from build123d import *

# Parameters (mm, degrees)
LUG_PLATE_PROFILE_SKETCH_R   = 7.5
LUG_PLATE_PROFILE_14MM_DEPTH = 14
CROSS_BLOCK_SKETCH_W         = 91
CROSS_BLOCK_SKETCH_H         = 84
CROSS_BLOCK_91X84_DEPTH      = 50
CENTRE_POCKET_SKETCH_W       = 55
CENTRE_POCKET_SKETCH_H       = 58
CENTRE_POCKET_55X58_DEPTH    = 50
CLEARANCE_CUT_SKETCH_R       = 8
CLEARANCE_CUT_DEPTH          = 172.161473469
LUG_PIN_HOLES_SKETCH_W       = 55
LUG_PIN_HOLES_SKETCH_H       = 28
LUG_PIN_HOLE_CUT_20MM_DEPTH  = 20
LUG_START                    = -50
SKETCH7_4_W                  = 55
SKETCH7_4_H                  = 28
LUG_PIN_HOLE_CUT_22MM_DEPTH  = 22


with BuildPart() as part:
    # Lug Plate Profile Sketch → Lug Plate Profile 14mm (new body)
    with BuildSketch(Plane.XY):
        Polygon((-94.388010718, 0), (95.611989282, 0), (95.611989282, 20), (70.611989282, 50), (-69.388010718, 50), (-94.388010718, 20), align=None)
        with Locations((-77.5, 15.791749187)):
            Circle(LUG_PLATE_PROFILE_SKETCH_R, mode=Mode.SUBTRACT)
        with Locations((77.5, 15.791749187)):
            Circle(LUG_PLATE_PROFILE_SKETCH_R, mode=Mode.SUBTRACT)
    extrude(amount=LUG_PLATE_PROFILE_14MM_DEPTH)

    # Cross Block Sketch → Cross Block 91x84 (add)
    with BuildSketch(Plane(origin=(0, 50, 0), x_dir=(1, 0, 0), z_dir=(0, 1, 0))):
        with Locations((0.611989282, 42)):
            Rectangle(CROSS_BLOCK_SKETCH_W, CROSS_BLOCK_SKETCH_H)
    extrude(amount=-CROSS_BLOCK_91X84_DEPTH)

    # Centre Pocket Sketch → Centre Pocket 55x58 (cut)
    with BuildSketch(Plane(origin=(0, 50, 0), x_dir=(1, 0, 0), z_dir=(0, 1, 0))):
        with Locations((0.611989282, 55)):
            Rectangle(CENTRE_POCKET_SKETCH_W, CENTRE_POCKET_SKETCH_H)
    extrude(amount=-CENTRE_POCKET_55X58_DEPTH, mode=Mode.SUBTRACT)

    # Clearance Cut Sketch → Clearance Cut (cut, through all)
    with BuildSketch(Plane(origin=(46.111989282, 0, 0), x_dir=(0, 0, -1), z_dir=(1, 0, 0))):
        with Locations(Location((44, 25, 0), (0, 0, 90))):
            Circle(CLEARANCE_CUT_SKETCH_R)
        with BuildLine():
            ThreePointArc((59.934024659, 50), (68.709034667, 25), (59.934024659, 0))
            Line((59.934024659, 0), (84, 0))
            Line((84, 0), (84, 50))
            Line((84, 50), (59.934024659, 50))
        make_face()
    extrude(amount=-CLEARANCE_CUT_DEPTH, mode=Mode.SUBTRACT)

    # Lug Pin Holes Sketch → Lug Pin Hole Cut 20mm (cut)
    with BuildSketch(Plane(origin=(0, 50, 0), x_dir=(1, 0, 0), z_dir=(0, 1, 0))):
        with Locations((0.611989282, 0)):
            Rectangle(LUG_PIN_HOLES_SKETCH_W, LUG_PIN_HOLES_SKETCH_H)
    extrude(amount=-LUG_PIN_HOLE_CUT_20MM_DEPTH, mode=Mode.SUBTRACT)

    # Sketch7_4 → Lug Pin Hole Cut 22mm (cut)
    with BuildSketch(Plane(origin=(0, 50, 0), x_dir=(1, 0, 0), z_dir=(0, 1, 0)).offset(LUG_START)):
        with Locations((0.611989282, 0)):
            Rectangle(SKETCH7_4_W, SKETCH7_4_H)
    extrude(amount=LUG_PIN_HOLE_CUT_22MM_DEPTH, mode=Mode.SUBTRACT)


solid = part.part
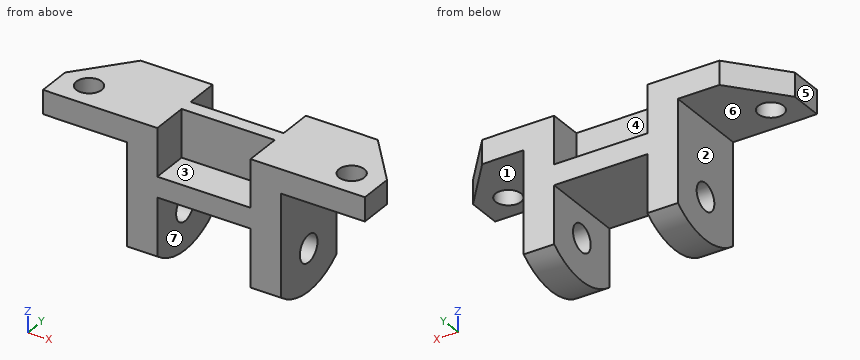
For this review, take the finished solid that the model builds, in its own axes (mm). Face numbers are marked on the shaded views. A direction names the side the tool comes from. Round coordinates to 2 decimals unless told otherwise and drop trailing zeros. Order: outer loops, then holes, each group sorted by start corner. A loop starts at its lowest first (then second) coordinate and runs counter-clockwise, first axis right, second up. Notation, with made-up numbers: (-9, 80) -> (42, 80) arc R24 cw to (42, 111) -> close; hole circle Ø8 at (40, 72). An arc over 180 degrees is marked (long way). Write item = value, one per line. Start each with the question number.
1) Take a section at C-C on y = 25. State the section outline as (x, z) points, plus the area to 3 significant figures.
2) Take a section at B-B on x = -77.5. State the section outline as (y, z) points, plus the area to 3 significant figures.
3) To check wall thickness, follow line 1 (X direction, y = 16, z = 2); line 2 (X direction, y = 45, z = -55); line 3 (Z direction, x = -31, y = 25). State the ranges of each line that lie inside material, in increasing order. Write a range as from..to.
4) The part is to be moulded in two halves that separate along X. For the marked faces 5, 6 and 7, say which applies: +X half, -X half, draft (parallel to the pull), parting line (faces both ways), or undercut.
5) Take a section at A-A on z = -44. State the section outline as (x, y) points, plus the area to 3 significant figures.
6) Insertion check: pin 1 (6 mm diameter, centred on x = 15.5, y = 36, fed in from -Z); pin 2 (10 mm diameter, centred on x = 3.5, y = 44, fed in from +Z); pin 3 (2 mm diameter, centred on y = 6.5, z = -2.5, fed in from +X); pin 4 (13 mm diameter, centred on y = 25, z = -44, fed in from +X). Each pin has a flat end and moves straight along its axis. Give the tip position at first contact, or say it passes through.
7) Tool access review of the marked faces 1, 2, 3 and 4: name each direction out of +Z, -Z, +X, -X, +Y, -Y from which nothing blocks a thin tool from reaching the whole face with its end or side.
8) Take a section at D-D on x = 19. State the section outline as (y, z) points, plus the area to 3 significant figures.
Verdict:
q1.outline = (-90.22, 0) -> (-44.89, 0) -> (-44.89, -36) -> (-26.89, -36) -> (-26.89, -26) -> (28.11, -26) -> (28.11, -36) -> (46.11, -36) -> (46.11, 0) -> (91.45, 0) -> (91.45, 14) -> (-90.22, 14) -> close; (-44.89, -68.71) -> (-26.89, -68.71) -> (-26.89, -52) -> (-44.89, -52) -> close; (28.11, -68.71) -> (46.11, -68.71) -> (46.11, -52) -> (28.11, -52) -> close
q1.area = 5,870 mm2
q2.outline = (0, 0) -> (8.29, 0) -> (8.29, 14) -> (0, 14) -> close; (23.29, 0) -> (40.27, 0) -> (40.27, 14) -> (23.29, 14) -> close
q2.area = 354 mm2
q3.line_1 = -94.39..-85, -70..-26.89, 28.11..70, 85..95.61
q3.line_2 = -44.89..-26.89, 28.11..46.11
q3.line_3 = -68.71..-52, -36..14
q4.face_5 = -X half
q4.face_6 = draft
q4.face_7 = undercut
q5.outline = (-44.89, 0) -> (-26.89, 0) -> (-26.89, 17) -> (-44.89, 17) -> close; (-44.89, 33) -> (-26.89, 33) -> (-26.89, 50) -> (-44.89, 50) -> close; (28.11, 0) -> (46.11, 0) -> (46.11, 17) -> (28.11, 17) -> close; (28.11, 33) -> (46.11, 33) -> (46.11, 50) -> (28.11, 50) -> close
q5.area = 1,220 mm2
q6.pin_1 = -26
q6.pin_2 = -14
q6.pin_3 = 46.11
q6.pin_4 = through
q7.face_1 = -Z, +X, +Y, -Y
q7.face_2 = -Z, -X, +Y, -Y
q7.face_3 = +Z, -Y
q7.face_4 = +Z, +Y
q8.outline = (0, -26) -> (50, -26) -> (50, -14) -> (30, -14) -> (30, 14) -> (22, 14) -> (22, -14) -> (0, -14) -> close
q8.area = 824 mm2
